The listing builds one solid part. Answer for the finished solid, in the listing's coordinates (mm). Face numbers are marked on the shaded views. A direction names the side the tool comes from. Give positions to 0.01 mm unless a question says otherwise; leave off trailing zeros. Order: outer loops, then holes, each group sorted by start corner. A loop starts at its lowest first (then second) coordinate and runs counter-clockwise, first axis right, second up.
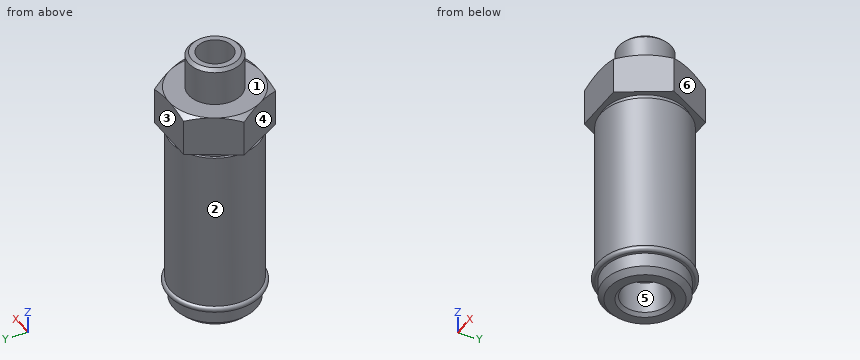
```python
from build123d import *

# Parameters (mm, degrees)
CUT_EXTRUDE_START   = -7.4
SKETCH_2_R          = 17
CUT_EXTRUDE_1_DEPTH = 7.4


with BuildPart() as part:
    # 草图1 → 旋转1 (revolve)
    with BuildSketch(Plane(origin=(0, 0, 0), x_dir=(0, 0, -1), z_dir=(1, 0, 0)), mode=Mode.PRIVATE) as revolve_1_sk:
        with BuildLine():
            Line((-26.4, 0), (-26.4, 3.242666667))
            Line((-26.4, 3.242666667), (-46.4, 3.242666667))
            Line((-46.4, 3.242666667), (-46.4, 4.283))
            Line((-46.4, 4.283), (-45.819, 4.864))
            Line((-45.819, 4.864), (-39.4, 4.864))
            Line((-39.4, 4.864), (-39.4, 8.5))
            Line((-39.4, 8.5), (-34.492522712, 17))
            Line((-34.492522712, 17), (-32, 17))
            Line((-32, 17), (-32, 7.65))
            Line((-32, 7.65), (-31, 7.65))
            Line((-31, 7.65), (-31, 8.15))
            Line((-31, 8.15), (-1.099431524, 8.15))
            ThreePointArc((-1.099431524, 8.15), (-0.537496769, 8.674857863), (0, 8.125))
            Line((0, 8.125), (0, 7.65))
            Line((0, 7.65), (2.6, 7.65))
            Line((2.6, 7.65), (3.6, 6.65))
            Line((3.6, 6.65), (3.6, 4.864))
            Line((3.6, 4.864), (3.019, 4.283))
            Line((3.019, 4.283), (-2.9, 4.283))
            Line((-2.9, 4.283), (-2.9, 0))
            Line((-2.9, 0), (-26.4, 0))
        make_face()
    revolve(revolve_1_sk.sketch.rotate(Axis((0, 0, -3.6), (0, 0, 1)), 180), axis=Axis((0, 0, -3.6), (0, 0, 1)))

    # 草图2 → 切除-拉伸1 (cut)
    with BuildSketch(Plane.XY.offset(39.4).offset(CUT_EXTRUDE_START)):
        Circle(SKETCH_2_R)
        Polygon((-4.907477288, -8.5), (4.907477288, -8.5), (9.814954576, 0), (4.907477288, 8.5), (-4.907477288, 8.5), (-9.814954576, 0), align=None, mode=Mode.SUBTRACT)
    extrude(amount=CUT_EXTRUDE_1_DEPTH, mode=Mode.SUBTRACT)


solid = part.part
```
1) Given P1, Ø6, axis at x = 0, z = 36, coming from the +Y side; P2, Ø2, axis at x = -5.5, z = 38, coming from the -Y side; P3, Ø2, axis at x = -0.5, z = 13, coming from the -Y side; P4, Ø5, axis at x = 0, y = -1, coming from the +Z side, each flat-ended and moving along its own axis, determine where each tip first touches the part or whether it passes through.
Geometry says:
P1: stops at y = 8.5
P2: stops at y = -8.5
P3: stops at y = -8.15
P4: stops at z = 46.4
2) Find section A-A (z = 34). Write down the section's boundary in (x, y), then the cut area to 3 significant figures.
Geometry says:
outline: (-9.81, 0) - (-4.91, -8.5) - (4.91, -8.5) - (9.81, 0) - (4.91, 8.5) - (-4.91, 8.5) - close; hole circle Ø6.49 at (0, 0)
area: 217 mm2
3) For a pull along Y with two mould halves and no side action, classify the marked faces 4, 5 and 6 as +Y half, -Y half, draft (parallel to the pull), parting line (faces both ways), or undercut.
Geometry says:
face 4: -Y half
face 5: undercut
face 6: +Y half
4) Find section B-B (z = 13). Write down the section's boundary in (x, y), then the cut area to 3 significant figures.
Geometry says:
outline: circle Ø16.3 at (0, 0)
area: 209 mm2
5) A tool of negligible diameter and unlimited length cuts with its end or side. For the marked faces 1, 2 and 3, from which of +Z, -Z, +X, -X, +Y, -Y can it reach the whole face along a straight path? Write none if from no direction.
Geometry says:
face 1: +Z
face 2: none
face 3: +Z, +X, -X, +Y
6) Straight lines are drawn through the part: probe 1 along X at (y, z) = (0, 41.75); probe 2 along X at (y, z) = (0, 1.6); probe 3 along Z at (x, y) = (-4, -7). For each, find the intervals that lie inside material, in ascending order.
Geometry says:
probe 1: x = -4.86 to -3.24, 3.24 to 4.86
probe 2: x = -8.15 to -4.28, 4.28 to 8.15
probe 3: z = 0 to 31, 32 to 39.4
7) Find section C-C (z = 40). Write down the section's boundary in (x, y), then the cut area to 3 significant figures.
Geometry says:
outline: circle Ø9.73 at (0, 0); hole circle Ø6.49 at (0, 0)
area: 41.3 mm2
